Work out the finished part from the listing and answer in its coordinate system (mm). A direction names the side the tool comes from. Coordinates: 2 decimals unless noted, no trailing zeros. Loops run counter-clockwise (first coordinate to the right, second up) from the corner with the lowest first, then second, coordinate; pieces in that order, holes last. Notation, with made-up numbers: (89, -11.5) -> (104, -11.5) arc R22 cw to (104, -2.5) -> close; hole circle Ø11 at (-6.75, 70.25). An arc over 180 degrees is marked (long way). Use a Markdown table: item, result.
from build123d import *


with BuildPart() as part:
    # 草图1 → 旋转1 (revolve)
    with BuildSketch(Plane.XY, mode=Mode.PRIVATE) as revolve_1_sk:
        Polygon((0, 0), (0, 2.0095), (0.4905, 2.5), (15, 2.5), (15, 2.065), (16.5, 2.065), (16.5, 2.5), (100.5, 2.5), (100.5, 8), (105.5, 8), (105.5, 0), align=None)
    revolve(revolve_1_sk.sketch.rotate(Axis((105.5, 0, 0), (-1, 0, 0)), 270), axis=Axis((105.5, 0, 0), (-1, 0, 0)))


solid = part.part
Q1. Consider line 1 (X direction, y = -2.25, z = 3.5); line 2 (X direction, y = -1.25, z = 1.75); line 3 (X direction, y = -1, z = 2). Determine where each line is inside the solid, lowest interval first. Write a range as [from, to].
Solved:
| item | result |
|---|---|
| line 1 | [100.5, 105.5] |
| line 2 | [0.14, 15], [16.5, 105.5] |
| line 3 | [0.23, 15], [16.5, 105.5] |
Q2. Section C-C on x = 48 is taken. Determine the outline of the cut face in (y, z).
Solved:
| item | result |
|---|---|
| outline | circle Ø5 at (0, 0) |
Q3. Given pin 1 Ø6 at (x, z) = (73.5, -3.5) entering from -Y; pin 2 Ø2 at (x, z) = (70, 0) entering from +Y; pin 3 Ø5 at (x, y) = (24.5, -3) entering from -Z, each flat-ended and moving along its own axis, determine where each tip first touches the part or whether it passes through.
Solved:
| item | result |
|---|---|
| pin 1 | y = -2.45 |
| pin 2 | y = 2.5 |
| pin 3 | z = -2.45 |
Q4. Section A-A on z = 0 is taken. Determine the outline of the cut face in (x, y) (1 decimal).
Solved:
| item | result |
|---|---|
| outline | (0, -2) -> (0.5, -2.5) -> (15, -2.5) -> (15, -2.1) -> (16.5, -2.1) -> (16.5, -2.5) -> (100.5, -2.5) -> (100.5, -8) -> (105.5, -8) -> (105.5, 8) -> (100.5, 8) -> (100.5, 2.5) -> (16.5, 2.5) -> (16.5, 2.1) -> (15, 2.1) -> (15, 2.5) -> (0.5, 2.5) -> (0, 2) -> close |
Q5. For faces 1 (the flat face through (0, 0, 0)), 2 (the cylindrical face through (15.76, -1.257, -1.639)), 3 (the cylindrical face through (7.85, -2.44, -0.54)), determine the directions among +Z, -Z, +X, -X, +Y, -Y from which every point of the face is accessible in a straight line to the end or side of a thin tool.
Solved:
| item | result |
|---|---|
| face 1 | +Z, -Z, -X, +Y, -Y |
| face 2 | none |
| face 3 | -X |
Q6. Section D-D on y = -4.75 is taken. Determine the outline of the cut face in (x, z), and give its area (3 significant figures).
Solved:
| item | result |
|---|---|
| outline | (100.5, -6.44) -> (105.5, -6.44) -> (105.5, 6.44) -> (100.5, 6.44) -> close |
| area | 64.4 mm² |
Q7. Determine the mould class of faces 4 (the cylindrical face through (103.04, -7.81, -1.73)), 5 (the flat face through (105.5, 0, 0)), 6 (the flat face through (15, 2, -1)), 7 (the flat face through (16.5, 2, 1)) for opening direction X: pulls with the +X half, pulls with the -X half, needs draft (parallel to the pull), parting line crosses it, or undercut.
Solved:
| item | result |
|---|---|
| face 4 | needs draft |
| face 5 | pulls with the +X half |
| face 6 | undercut |
| face 7 | undercut |
